The listing builds one solid part. Answer for the finished solid, in the listing's coordinates (mm). A direction names the side the tool comes from. Coordinates: 2 decimals unless noted, no trailing zeros. Write each loop counter-clockwise with the first axis right and the second up, starting at its lowest first coordinate (ties: lowest second). Pieces come first, ordered by that corner, then holes. Notation, with made-up numbers: M -11.5,77 L 14.5,77 A24 ccw 14.5,112 Z; hole C 46,-8 d2. An arc over 180 degrees is marked long. Answer as CSV lines item,"result". Start each with the question number.
```python
from build123d import *

# Parameters (mm, degrees)
GB_6728_1986_RECTANGULAR_HOLLOW_SECTION_DEPTH = 1590


with BuildPart() as part:
    # Sketch14 → Gb/6728-1986 rectangular hollow section 060 X 40 X 3 (new body)
    with BuildSketch(Plane(origin=(0, 0, 0), x_dir=(-1, 0, 0), z_dir=(0, 0, -1))):
        with BuildLine():
            Line((-14, -30), (14, -30))
            ThreePointArc((14, -30), (18.242640687, -28.242640687), (20, -24))
            Line((20, -24), (20, 24))
            ThreePointArc((20, 24), (18.242640687, 28.242640687), (14, 30))
            Line((14, 30), (-14, 30))
            ThreePointArc((-14, 30), (-18.242640687, 28.242640687), (-20, 24))
            Line((-20, 24), (-20, -24))
            ThreePointArc((-20, -24), (-18.242640687, -28.242640687), (-14, -30))
        make_face()
        with BuildLine():
            Line((-14, -27), (14, -27))
            ThreePointArc((14, -27), (16.121320344, -26.121320344), (17, -24))
            Line((17, -24), (17, 24))
            ThreePointArc((17, 24), (16.121320344, 26.121320344), (14, 27))
            Line((14, 27), (-14, 27))
            ThreePointArc((-14, 27), (-16.121320344, 26.121320344), (-17, 24))
            Line((-17, 24), (-17, -24))
            ThreePointArc((-17, -24), (-16.121320344, -26.121320344), (-14, -27))
        make_face(mode=Mode.SUBTRACT)
    extrude(amount=GB_6728_1986_RECTANGULAR_HOLLOW_SECTION_DEPTH)


solid = part.part
```
1) The part is cut by section B-B (z = -274). Determine the outline of the cut face in (x, y).
2) The part is cut by section A-A (x = -3). Determine the outline of the cut face in (y, z).
3) The part is cut by section C-C (y = -5). Determine the outline of the cut face in (x, z).
4) For a pull along X with two mould halves and no side action, classify faces 1 (the face through (-20, 0, -784)), 2 (the face through (0, -30, -784)), 3 (the face through (0, 27, -784)), 4 (the face through (20, 0, -784)) as +X half, -X half, draft (parallel to the pull), parting line (faces both ways), or undercut.
5) Find the intervals of material crossed by line 1 (X direction, y = -20, z = -1053); line 2 (Y direction, x = 5, z = -592); line 3 (X direction, y = 25, z = -362.5), in increasing order. Write a range as from..to.
6) This flat-tipped pin is pushed along its axis until it touches: P1, Ø1, axis at x = 15, z = -284.5, coming from the +Y side. Where does it stop, or does it pass through?
7) Which of the six approach directions +Z, -Z, +X, -X, +Y, -Y give full straight-line access (tool end or side, diameter ignored) to faces 5 (the face through (-17, 0, -784)), 6 (the face through (0, 30, -784))?
Completed:
1,outline,"M -20,-24 A6 ccw -14,-30 L 14,-30 A6 ccw 20,-24 L 20,24 A6 ccw 14,30 L -14,30 A6 ccw -20,24 Z; hole M -17,-24 A3 ccw -14,-27 L 14,-27 A3 ccw 17,-24 L 17,24 A3 ccw 14,27 L -14,27 A3 ccw -17,24 Z"
2,outline,"M -30,-1590 L -27,-1590 L -27,0 L -30,0 Z; M 27,-1590 L 30,-1590 L 30,0 L 27,0 Z"
3,outline,"M -20,-1590 L -17,-1590 L -17,0 L -20,0 Z; M 17,-1590 L 20,-1590 L 20,0 L 17,0 Z"
4,face 1,"-X half"
4,face 2,"draft"
4,face 3,"undercut"
4,face 4,"+X half"
5,line 1,"-20..-17, 17..20"
5,line 2,"-30..-27, 27..30"
5,line 3,"-19.92..-16.83, 16.83..19.92"
6,P1,"y = 29.98"
7,face 5,"+Z, -Z"
7,face 6,"+Z, -Z, +X, -X, +Y"
